Can you work these out from the drawing? Everything is in mm from the part's minimum corner. Give positions to 0.01 mm unless a question says otherwise; leave off trailing zeros. Order: outer loops, then holes, each group sorted by start corner. A loop starts at its lowest first (then second) coordinate and runs counter-clockwise, first axis right, second up. Notation, with made-up numbers: (72.25, 66.5) - (115.25, 66.5) arc R8 ccw to (115.25, 70.5) - close; hole circle Ø1 at (83, -30.75). An arc over 180 degrees is marked (long way). Answer as a JSON object with one key per item and string values.
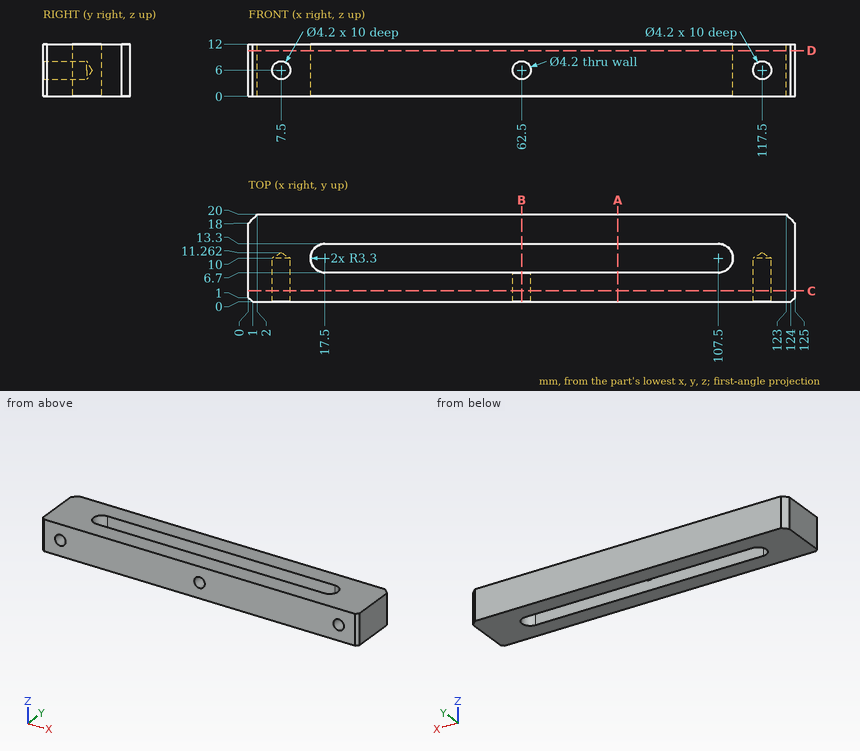
Q1. I need wall thicknesses on L1, parallel to Y at x = 76, z = 8.5; L2, parallel to Z at x = 7.5, y = 3.75; L3, parallel to X at y = 13, z = 2.75 (1 decimal). Which ranges of each line are inside material? Lowest first, please.
Recorded:
{"L1": "y = 0 to 6.7, 13.3 to 20", "L2": "z = 0 to 3.9, 8.1 to 12", "L3": "x = 0 to 16.1, 108.9 to 125"}
Q2. If we section it at B-B, the plane x = 62.5: Please give me the cut outline in (y, z).
Recorded:
{"outline": "(0, 0) - (6.7, 0) - (6.7, 3.9) - (0, 3.9) - close; (0, 8.1) - (6.7, 8.1) - (6.7, 12) - (0, 12) - close; (13.3, 0) - (20, 0) - (20, 12) - (13.3, 12) - close"}
Q3. If we section it at A-A, the plane x = 84.5: Please give me the cut outline in (y, z).
Recorded:
{"outline": "(0, 0) - (6.7, 0) - (6.7, 12) - (0, 12) - close; (13.3, 0) - (20, 0) - (20, 12) - (13.3, 12) - close"}
Q4. I'm going to push a flat-ended pin straight in: pin 1 Ø4 at (x, z) = (62.5, 6) entering from -Y. Where does the tip first touch, or does it pass through?
Recorded:
{"pin 1": "stops at y = 13.3"}
Q5. If we section it at C-C, the plane y = 2.5: Please give me the cut outline in (x, z), then the cut area to 3 significant figures.
Recorded:
{"outline": "(0, 0) - (125, 0) - (125, 12) - (0, 12) - close; hole circle Ø4.2 at (7.5, 6); hole circle Ø4.2 at (62.5, 6); hole circle Ø4.2 at (117.5, 6)", "area": "1,460 mm^2"}
Q6. If we section it at D-D, the plane z = 10.5: Please give me the cut outline in (x, y).
Recorded:
{"outline": "(0, 1) - (1, 0) - (124, 0) - (125, 1) - (125, 18) - (123, 20) - (2, 20) - (0, 18) - close; hole (17.5, 6.7) - (107.5, 6.7) arc R3.3 ccw to (107.5, 13.3) - (17.5, 13.3) arc R3.3 ccw to start"}
